```python
from build123d import *

# Parameters (mm, degrees)
FLANGE_STEP_A_DEPTH  = 10
FLANGE_RIB_SKETCH_W  = 10
FLANGE_RIB_SKETCH_H  = 10
FLANGE_RIB_DEPTH     = 10
CLAMP_BAND_DEPTH     = 65
FLANGE_STEP_B_DEPTH  = 10
FLANGE_WEB_DEPTH     = 65
MOUNTING_LUG_1_DEPTH = 10
MOUNTING_LUG_2_DEPTH = 10
BOLT_HOLE_1_SKETCH_R = 7.5
BOLT_HOLE_1_15_DEPTH = 20
BOLT_HOLE_2_SKETCH_R = 7.5
BOLT_HOLE_2_15_DEPTH = 20


with BuildPart() as part:
    # Flange Step A Sketch → Flange Step A (new body)
    with BuildSketch(Plane.XY):
        with BuildLine():
            Line((0, 10), (-40, 10))
            ThreePointArc((-40, 10), (-43.535533906, 11.464466094), (-45, 15))
            Line((-45, 15), (-45, 70))
            ThreePointArc((-45, 70), (-43.535533906, 73.535533906), (-40, 75))
            Line((-40, 75), (0, 75))
            Line((0, 75), (0, 10))
        make_face()
    extrude(amount=FLANGE_STEP_A_DEPTH)

    # Flange Rib Sketch → Flange Rib (add)
    with BuildSketch(Plane.XY.offset(10)):
        with Locations((-5, 70)):
            Rectangle(FLANGE_RIB_SKETCH_W, FLANGE_RIB_SKETCH_H)
        with Locations((-5, 15)):
            Rectangle(FLANGE_RIB_SKETCH_W, FLANGE_RIB_SKETCH_H)
    extrude(amount=FLANGE_RIB_DEPTH)

    # Clamp Band Sketch → Clamp Band (add)
    with BuildSketch(Plane(origin=(0, 75, 0), x_dir=(1, 0, 0), z_dir=(0, 1, 0))):
        with BuildLine():
            Line((-10.624085248, 0), (0, 0))
            ThreePointArc((0, 0), (60, 60), (120, 0))
            Line((120, 0), (130.624085248, 0))
            ThreePointArc((130.624085248, 0), (60, 70.624085248), (-10.624085248, 0))
        make_face()
    extrude(amount=-CLAMP_BAND_DEPTH)



with BuildPart() as body_2:
    # Flange Step B Sketch → Flange Step B (new body)
    with BuildSketch(Plane.XY):
        with BuildLine():
            Line((130.624085248, 75), (165.624085248, 75))
            ThreePointArc((165.624085248, 75), (169.159619153, 73.535533906), (170.624085248, 70))
            Line((170.624085248, 70), (170.624085248, 15))
            ThreePointArc((170.624085248, 15), (169.159619153, 11.464466094), (165.624085248, 10))
            Line((165.624085248, 10), (130.624085248, 10))
            Line((130.624085248, 10), (130.624085248, 75))
        make_face()
    extrude(amount=FLANGE_STEP_B_DEPTH)


with BuildPart() as part_1:
    add(part.part)

    add(body_2.part)  # Flange Web merges body 2
    # Flange Web Sketch → Flange Web (add)
    with BuildSketch(Plane(origin=(0, 75, 0), x_dir=(1, 0, 0), z_dir=(0, 1, 0))):
        Polygon((130.624085248, 0), (130.624085248, -20), (120.624085248, -20), (120, 0), align=None)
    extrude(amount=-FLANGE_WEB_DEPTH)

    # Mounting Lug 1 Sketch → Mounting Lug 1 (add)
    with BuildSketch(Plane(origin=(0, 0, 0), x_dir=(-1, 0, 0), z_dir=(0, 0, -1))):
        with BuildLine():
            Line((-130.624085248, 60), (-145.624085248, 60))
            ThreePointArc((-145.624085248, 60), (-163.124085248, 42.5), (-145.624085248, 25))
            Line((-145.624085248, 25), (-130.624085248, 25))
            Line((-130.624085248, 25), (-130.624085248, 60))
        make_face()
    extrude(amount=MOUNTING_LUG_1_DEPTH)

    # Mounting Lug 2 Sketch → Mounting Lug 2 (add)
    with BuildSketch(Plane(origin=(0, 0, 0), x_dir=(-1, 0, 0), z_dir=(0, 0, -1))):
        with BuildLine():
            Line((10.624085248, 60), (10.624085248, 25))
            Line((10.624085248, 25), (20.624085248, 25))
            ThreePointArc((20.624085248, 25), (38.124085248, 42.5), (20.624085248, 60))
            Line((20.624085248, 60), (10.624085248, 60))
        make_face()
    extrude(amount=MOUNTING_LUG_2_DEPTH)

    # Bolt Hole 1 Sketch → Bolt Hole 1 Ø15 (cut)
    with BuildSketch(Plane(origin=(0, 0, -10), x_dir=(-1, 0, 0), z_dir=(0, 0, -1))):
        with Locations((-145.624085248, 42.5)):
            Circle(BOLT_HOLE_1_SKETCH_R)
    extrude(amount=-BOLT_HOLE_1_15_DEPTH, mode=Mode.SUBTRACT)

    # Bolt Hole 2 Sketch → Bolt Hole 2 Ø15 (cut)
    with BuildSketch(Plane(origin=(0, 0, -10), x_dir=(-1, 0, 0), z_dir=(0, 0, -1))):
        with Locations((22.530823522, 43.946489257)):
            Circle(BOLT_HOLE_2_SKETCH_R)
    extrude(amount=-BOLT_HOLE_2_15_DEPTH, mode=Mode.SUBTRACT)


solid = part_1.part
```
Here's how the part is built. I have some questions about the finished solid (model axes, mm). A direction names the side the tool comes from. Coordinates: 2 decimals unless noted, no trailing zeros. Order: outer loops, then holes, each group sorted by start corner. A loop starts at its lowest first (then second) coordinate and runs counter-clockwise, first axis right, second up. Notation, with made-up numbers: M 60,-3 L 114,-3 A22 ccw 114,31 Z; hole C 49.25,40.25 d4. An arc over 180 degrees is marked long. Answer as a JSON object with one key per item and string values. Group by question number.
(1) Suppose I cut it at A-A, the plane z = -30. Please give me the cut outline in (x, y).
(2) Which directions (+Z, -Z, +X, -X, +Y, -Y) give clear straight access to the entire face, cutting with the end or side of a thin tool? Please do faces 4 (the face through (138, 25, -5)), 5 (the face through (-5, 20, 15)), 6 (the face through (147.1, 34.97, -10)), 7 (the face through (-10.624, 43, -5)).
(3) Suppose I cut it at D-D, the plane x = 82. Please give me the cut outline in (y, z).
(4) For pin 1 (3 mm diameter, centred on x = 91, y = 42.5, fed in from -Z); pin 2 (8 mm diameter, centred on x = 23.5, y = 29, fed in from +Z); pin 3 (11 mm diameter, centred on y = 55, z = 16.5, fed in from +X), each with a flat end and sliding along its axis, tell me the tip position at first contact or that it passes through.
(5) Suppose I cut it at B-B, the plane z = 6.5. Please give me the cut outline in (x, y).
(6) If we mould it in two halves opening along Y, with no side actions, what happens to faces 1 (the face through (170.624, 43, 5)), 2 (the face through (-5, 65, 15)), 3 (the face through (-44, 73, 5))? For each: released by +Y, released by -Y, zero draft, split by the parting line, or undercut.
(7) I need wall thicknesses on probe 1 along Z at (x, y) = (145.5, 34.5); probe 2 along X at (y, z) = (42, 6); probe 3 along X at (y, z) = (42, 2). Which ranges of each line are inside material? Lowest first, please.
(8) Suppose I cut it at C-C, the plane y = 54.5. Please give me the cut outline in (x, z), then the cut area to 3 significant figures.
Values found:
{
 "1": {"outline": "M -3.94,10 L 8.04,10 L 8.04,75 L -3.94,75 Z; M 111.96,10 L 123.94,10 L 123.94,75 L 111.96,75 Z"},
 "2": {"face 4": "-Z, +X, -Y", "face 5": "+Z, -X", "face 6": "-Z, +X, +Y, -Y", "face 7": "none"},
 "3": {"outline": "M 10,-67.11 L 75,-67.11 L 75,-55.82 L 10,-55.82 Z"},
 "4": {"pin 1": "stops at z = -64.17", "pin 2": "stops at z = -44.27", "pin 3": "stops at x = 130.62"},
 "5": {"outline": "M -45,15 A5 ccw -40,10 L 0,10 L 0,75 L -40,75 A5 ccw -45,70 Z; M 120.2,10 L 165.62,10 A5 ccw 170.62,15 L 170.62,70 A5 ccw 165.62,75 L 120.2,75 Z; hole C -22.53,43.95 d15; hole C 145.62,42.5 d15"},
 "6": {"face 1": "zero draft", "face 2": "undercut", "face 3": "released by +Y"},
 "7": {"probe 1": "z = -10 to 10", "probe 2": "x = -45 to -29.77, -15.29 to 0, 120.19 to 138.14, 153.11 to 170.62", "probe 3": "x = -45 to -29.77, -15.29 to 0, 120.06 to 138.14, 153.11 to 170.62"},
 "8": {"outline": "M -45,0 L -33.36,0 L -33.36,-10 L -10.62,-10 L -10.62,0 A70.62 ccw 130.62,0 L 130.62,-10 L 158.36,-10 L 158.36,0 L 170.62,0 L 170.62,10 L 130.62,10 L 130.62,20 L 120.62,20 L 120,0 A60 cw 0,0 L 0,10 L -45,10 Z", "area": "3,740 mm^2"}
}
